Read the model definition and answer for the solid it produces. Units are mm, in the model's axes. A direction names the side the tool comes from. Give positions to 0.01 mm unless a question says otherwise; leave off trailing zeros. Loops run counter-clockwise (first coordinate to the right, second up) from the corner with the lowest first, then second, coordinate; pieces in that order, holes last. Notation, with made-up numbers: (62.25, 66.5) - (116.25, 66.5) arc R9 ccw to (116.25, 71.5) - close; hole circle Ø1 at (89, -28.5). An arc over 180 degrees is marked (long way). Use a Markdown table: item, result. Add a question column.
Item 1: Each of these flat-tipped pins is pushed along its axis until it touches: P1, Ø12, axis at x = -15, z = 11.5, coming from the +Y side; P2, Ø10, axis at x = -16, z = -7, coming from the -Y side; P3, Ø1, axis at x = -5.5, z = -15, coming from the -Y side. Where does it stop, or does it pass through?
Item 2: Which of the six approach directions +Z, -Z, +X, -X, +Y, -Y give full straight-line access (tool end or side, diameter ignored) to faces 1 (the face through (-34.83, 15.24, 6.32)), 2 (the face through (-13, 0, 18)), 3 (the face through (-48, -3, 10))?
Item 3: Consider probe 1 along Z at (x, y) = (-30, 0); probe 2 along Z at (x, y) = (-15, 0); probe 3 along Y at (x, z) = (-12, 0). Determine where each line is inside the solid, lowest interval first. Write a range as [from, to].
Item 4: A cutting plane is placed at A-A (z = 0). Determine the outline of the cut face in (x, y).
Item 5: For a pull along Y with two mould halves and no side action, classify faces 4 (the face through (-17.93, -4.336, 19.524)), 5 (the face through (-34.89, -2.17, -9.76)), 6 (the face through (-23, -2.9, -16.4)) as +Y half, -Y half, draft (parallel to the pull), parting line (faces both ways), or undercut.
Item 6: A cutting plane is placed at B-B (x = -30). Determine the outline of the cut face in (y, z).
Item 7: A cutting plane is placed at C-C (y = 18.5). Determine the outline of the cut face in (x, z), plus the area to 3 significant figures.
Item 8: A cutting plane is placed at D-D (x = -11). Determine the outline of the cut face in (y, z).
from build123d import *

# Parameters (mm, degrees)
SKETCH2_R                  = 10
CUT_EXTRUDE1_DEPTH         = 56.713553109
M22X1_5_TAPPED_HOLE2_D     = 20.5
M22X1_5_TAPPED_HOLE2_DEPTH = 22
M22X1_5_TAPPED_HOLE2_TIP   = 6.158821345


with BuildPart() as part:
    # Sketch1 → Revolve1 (revolve)
    with BuildSketch(Plane.XY):
        Polygon((-48, 0), (-48, 15.5), (-47, 16.5), (-23, 16.5), (-23, 20), (-13, 20), (-13, 17.5), (0, 17.5), (0, 0), align=None)
    revolve(axis=Axis((0, 0, 0), (-1, 0, 0)))

    # Sketch2 → Cut-Extrude1 (cut, through all)
    with BuildSketch(Plane(origin=(0, 0, 0), x_dir=(0, 0, -1), z_dir=(1, 0, 0))):
        with Locations(Location((0, 0, 0), (0, 0, 90))):
            Circle(SKETCH2_R)
    extrude(amount=-CUT_EXTRUDE1_DEPTH, mode=Mode.SUBTRACT)

    # M22x1.5 Tapped Hole2
    with Locations(Plane(origin=(0, 0, 0), x_dir=(0, 0, -1), z_dir=(1, 0, 0))):
        with Locations((0, 0)):
            Hole(M22X1_5_TAPPED_HOLE2_D / 2, depth=M22X1_5_TAPPED_HOLE2_DEPTH)
            with Locations((0, 0, -(M22X1_5_TAPPED_HOLE2_DEPTH + M22X1_5_TAPPED_HOLE2_TIP / 2))):  # 118° drill point
                Cone(0, M22X1_5_TAPPED_HOLE2_D / 2, M22X1_5_TAPPED_HOLE2_TIP, mode=Mode.SUBTRACT)


solid = part.part
Geometry says:
| question | item | result |
|---|---|---|
| 1 | P1 | y = 19.23 |
| 1 | P2 | y = -19.9 |
| 1 | P3 | y = -9.8 |
| 2 | face 1 | -X |
| 2 | face 2 | +X |
| 2 | face 3 | +Z, -Z, -X, +Y, -Y |
| 3 | probe 1 | [-16.5, -10], [10, 16.5] |
| 3 | probe 2 | [-20, -10.25], [10.25, 20] |
| 3 | probe 3 | [-17.5, -10.25], [10.25, 17.5] |
| 4 | outline | (-48, -15.5) - (-47, -16.5) - (-23, -16.5) - (-23, -20) - (-13, -20) - (-13, -17.5) - (0, -17.5) - (0, -10.25) - (-22, -10.25) - (-22.15, -10) - (-48, -10) - close; (-48, 10) - (-22.15, 10) - (-22, 10.25) - (0, 10.25) - (0, 17.5) - (-13, 17.5) - (-13, 20) - (-23, 20) - (-23, 16.5) - (-47, 16.5) - (-48, 15.5) - close |
| 5 | face 4 | parting line |
| 5 | face 5 | undercut |
| 5 | face 6 | draft |
| 6 | outline | circle Ø33 at (0, 0); hole circle Ø20 at (0, 0) |
| 7 | outline | (-23, -7.6) - (-13, -7.6) - (-13, 7.6) - (-23, 7.6) - close |
| 7 | area | 152 mm² |
| 8 | outline | circle Ø35 at (0, 0); hole circle Ø20.5 at (0, 0) |
